```python
from build123d import *

# Parameters (mm, degrees)
SKETCH2_R           = 1.5
BOSS_EXTRUDE1_DEPTH = 2


with BuildPart() as part:
    # Sketch2 → Boss-Extrude1 (new body)
    with BuildSketch(Plane(origin=(0, 0, 0), x_dir=(1, 0, 0), z_dir=(0, 1, 0))):
        with BuildLine():
            Line((-14.953942403, -20.676544339), (-13.710907235, -18.957822206))
            ThreePointArc((-13.710907235, -18.957822206), (-8.367273859, -17.591450428), (-6.055414365, -22.599114073))
            Line((-6.055414365, -22.599114073), (-7.272815167, -27.142515719))
            ThreePointArc((-7.272815167, -27.142515719), (0, 28.1), (7.272815167, -27.142515719))
            Line((7.272815167, -27.142515719), (6.055414365, -22.599114073))
            ThreePointArc((6.055414365, -22.599114073), (8.367273859, -17.591450428), (13.710907235, -18.957822206))
            Line((13.710907235, -18.957822206), (14.953942403, -20.676544339))
            ThreePointArc((14.953942403, -20.676544339), (0, 23.4), (-14.953942403, -20.676544339))
        make_face()
        with Locations(Location((-10.218554677, -21.483603988, 0), (0, 0, 270))):
            Circle(SKETCH2_R, mode=Mode.SUBTRACT)
        with Locations(Location((10.218554677, -21.483603988, 0), (0, 0, 90))):
            Circle(SKETCH2_R, mode=Mode.SUBTRACT)
    extrude(amount=BOSS_EXTRUDE1_DEPTH)


solid = part.part
```
Geometry check sheet. Reference: the model listing, model coordinates, mm. A direction names the side the tool comes from. Coordinates: 2 decimals unless noted, no trailing zeros. Order: outer loops, then holes, each group sorted by start corner. A loop starts at its lowest first (then second) coordinate and runs counter-clockwise, first axis right, second up. Notation, with made-up numbers: M 25.25,81.25 L 41.25,81.25 A18 ccw 41.25,102.25 Z; hole C 65.5,72 d4. An arc over 180 degrees is marked long. Answer as a JSON object with one key per item and string values.
Q1. Release check for a two-part mould opening along X. For faces 4 (the flat face through (-8, 0, 18)), 5 (the flat face through (-14.34, 0.99, 19.83)), 6 (the cylindrical face through (-1.133, 0.986, -28.077)) record: released by +X, released by -X, zero draft, split by the parting line, or undercut.
Results are:
{"face 4": "zero draft", "face 5": "undercut", "face 6": "split by the parting line"}
Q2. Tool access check on faces 1 (the flat face through (6.67, 0.99, 24.9)), 2 (the flat face through (14.324, 0.986, 19.805)), 3 (the flat face through (-8, 2, 18)). Record the directions out of +Z, -Z, +X, -X, +Y, -Y that give a thin tool (end or side, any length) a straight path to the whole face; none if there is none.
Results are:
{"face 1": "+Z, +Y, -Y", "face 2": "+Y, -Y", "face 3": "+Z, -Z, +X, -X, +Y"}
Q3. Cross-section at B-B on x = 21.5. Record the cut outline in (y, z).
Results are:
{"outline": "M 0,-18.09 L 2,-18.09 L 2,-10.73 L 0,-10.73 Z; M 0,13.08 L 2,13.08 L 2,18.09 L 0,18.09 Z"}
Q4. Cross-section at A-A on z = -19. Record the cut outline in (x, y).
Results are:
{"outline": "M -20.7,0 L -14.03,0 L -14.03,2 L -20.7,2 Z; M 14.03,0 L 20.7,0 L 20.7,2 L 14.03,2 Z"}
Q5. Cross-section at D-D on x = 0. Record the cut outline in (y, z), and give its area (3 significant figures).
Results are:
{"outline": "M 0,-28.1 L 2,-28.1 L 2,-23.4 L 0,-23.4 Z", "area": "9.40 mm²"}
Q6. Scan lines: line 1 (X direction, y = 1, z = 18); line 2 (Z direction, x = -11, y = 0.3); line 3 (Z direction, x = -10, y = 1.45). Record each from-to range of solid material in increasing order.
Results are:
{"line 1": "x = -21.58 to -17.91, -12.76 to -7.68, 7.68 to 12.76, 17.91 to 21.58", "line 2": "z = -25.86 to -20.8, 17.25 to 20.2, 22.76 to 25.86", "line 3": "z = -26.26 to -21.27, 17.18 to 20, 22.97 to 26.26"}
Q7. Depth check by flat-ended pin: pin 1 Ø3.5 at (x, z) = (-10.22, 21.48) entering from +Y; pin 2 Ø1 at (y, z) = (0.5, 17.5) entering from +X. Enter the tip coordinate at first touch or a pass-through.
Results are:
{"pin 1": "stops at y = 2", "pin 2": "stops at x = 22.37"}
Q8. Cross-section at C-C on y = 1.65. Record the cut outline in (x, z) (3 decimals), and give its area (3 significant figures).
Results are:
{"outline": "M -14.954,20.677 L -13.711,18.958 A4.31 ccw -6.055,22.599 L -7.273,27.143 A28.1 ccw long 7.273,27.143 L 6.055,22.599 A4.31 ccw 13.711,18.958 L 14.954,20.677 A24.575 cw long Z; hole C -10.219,21.484 d3; hole C 10.219,21.484 d3", "area": "625 mm²"}
